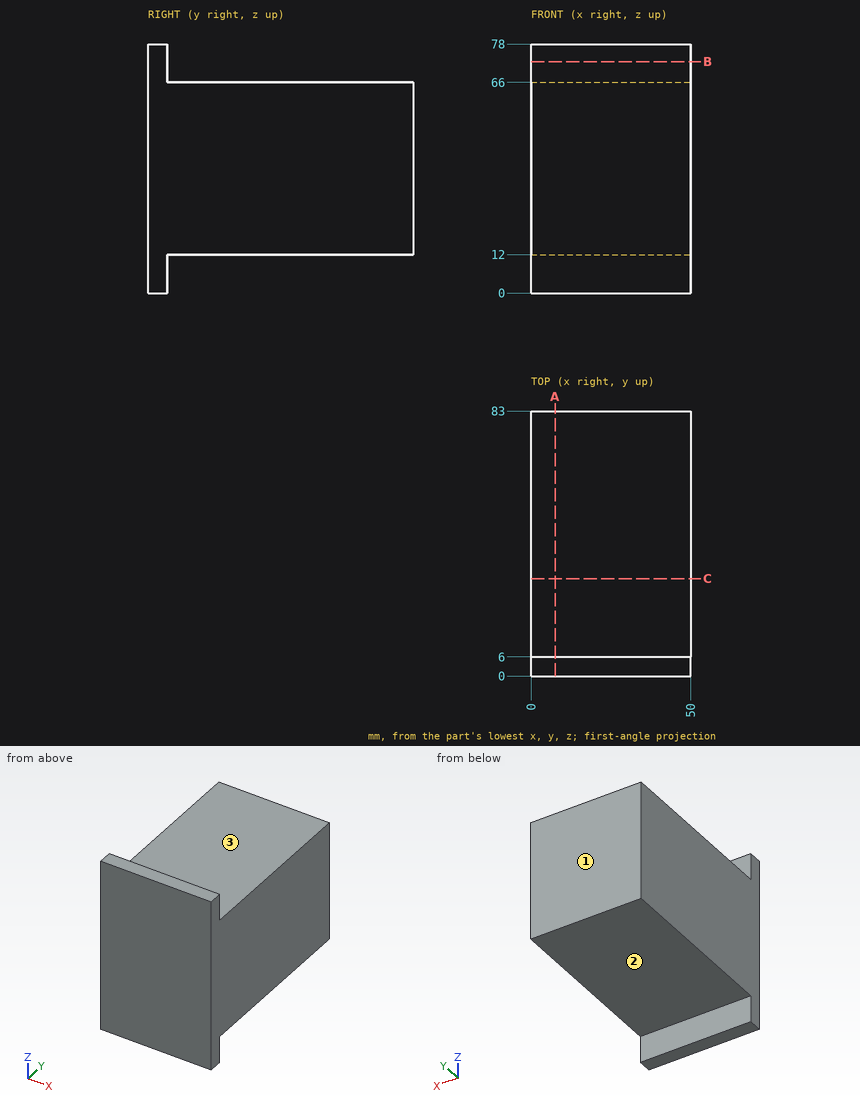
Study the drawing (mm; zero at the part's minimum x, y, z) and answer. A direction names the side the tool comes from. Give positions to 0.01 mm unless a question says otherwise; leave off trailing zeros. Loops run counter-clockwise (first coordinate to the right, second up) from the corner with the lowest first, then second, coordinate; pieces in that order, holes last. Notation, with made-up numbers: (-34, 52) - (25, 52) arc R26 cw to (25, 69) - close; hole circle Ø5 at (-34.5, 20). An arc over 180 degrees is marked (long way). Answer as CSV lines item,"result". Start each with the question number.
1) Which of the six approach directions +Z, -Z, +X, -X, +Y, -Y give full straight-line access (tool end or side, diameter ignored) to the marked faces 1, 2 and 3?
2) Find section A-A (x = 7.5). Write down the section's boundary in (y, z), then the cut area to 3 significant figures.
3) Straight lines are drawn through the part: L1, parallel to Z at x = 24, y = 53; L2, parallel to Y at x = 13, z = 11.5. For each, find the intervals that lie inside material, in ascending order. Write a range as from..to.
4) Each of these flat-tipped pins is pushed along its axis until it touches: pin 1 Ø2 at (x, y) = (27, 21) entering from -Z; pin 2 Ø6 at (x, z) = (18.5, 74.5) entering from +Y; pin 3 Ø25 at (x, y) = (16, 34) entering from +Z. Where does it stop, or does it pass through?
5) Find section C-C (y = 30.5). Write down the section's boundary in (x, z), then the cut area to 3 significant figures.
6) Find section B-B (z = 72.5). Write down the section's boundary in (x, y), then the cut area to 3 significant figures.
Findings below:
1,face 1,"+Z, -Z, +X, -X, +Y"
1,face 2,"-Z, +X, -X, +Y"
1,face 3,"+Z, +X, -X, +Y"
2,outline,"(0, 0) - (6, 0) - (6, 12) - (83, 12) - (83, 66) - (6, 66) - (6, 78) - (0, 78) - close"
2,area,"4,630 mm^2"
3,L1,"12..66"
3,L2,"0..6"
4,pin 1,"z = 12"
4,pin 2,"y = 6"
4,pin 3,"z = 66"
5,outline,"(0, 12) - (50, 12) - (50, 66) - (0, 66) - close"
5,area,"2,700 mm^2"
6,outline,"(0, 0) - (50, 0) - (50, 6) - (0, 6) - close"
6,area,"300 mm^2"
